from build123d import *

# Parameters (mm, degrees)
ROD_BODY_SKETCH_W                = 95
ROD_BODY_SKETCH_H                = 30
ROD_BODY_30X95_DEPTH             = 20
MOUNTING_PLATE_SKETCH_W          = 50
MOUNTING_PLATE_SKETCH_H          = 90
MOUNTING_PLATE_12MM_DEPTH        = 12
EYE_BOSS_DEPTH                   = 7.5
EYE_HOLE_SKETCH_R                = 12.5
EYE_HOLE_25_DEPTH                = 15
MOUNTING_SLOTS_2X10_DEPTH        = 138.095769446
PLATE_CORNER_CHAMFERS_10X45_SIZE = 10


with BuildPart() as part:
    # Rod Body Sketch → Rod Body 30x95 (new, symmetric)
    with BuildSketch(Plane.XY):
        Rectangle(ROD_BODY_SKETCH_W, ROD_BODY_SKETCH_H)
    extrude(amount=ROD_BODY_30X95_DEPTH, both=True)

    # Mounting Plate Sketch → Mounting Plate 12mm (add)
    with BuildSketch(Plane(origin=(0, 15, 0), x_dir=(1, 0, 0), z_dir=(0, 1, 0))):
        with Locations((-22.5, 0)):
            Rectangle(MOUNTING_PLATE_SKETCH_W, MOUNTING_PLATE_SKETCH_H)
    extrude(amount=MOUNTING_PLATE_12MM_DEPTH)

    # Eye Boss Sketch → Eye Boss (add, symmetric)
    with BuildSketch(Plane.XY):
        with BuildLine():
            Line((92.5, -15), (47.5, -15))
            Line((47.5, -15), (47.5, 15))
            Line((47.5, 15), (62.5, 15))
            ThreePointArc((62.5, 15), (113.713203436, 36.213203436), (92.5, -15))
        make_face()
    extrude(amount=EYE_BOSS_DEPTH, both=True)

    # Eye Hole Sketch → Eye Hole Ø25 (cut)
    with BuildSketch(Plane.XY.offset(7.5)):
        with Locations((92.5, 15)):
            Circle(EYE_HOLE_SKETCH_R)
    extrude(amount=-EYE_HOLE_25_DEPTH, mode=Mode.SUBTRACT)

    # Mounting Slots Sketch → Mounting Slots 2x10 (cut, through all)
    with BuildSketch(Plane(origin=(0, 27, 0), x_dir=(1, 0, 0), z_dir=(0, 1, 0))):
        with BuildLine():
            Line((-27.5, 20), (-27.5, 45))
            Line((-27.5, 45), (-17.5, 45))
            Line((-17.5, 45), (-17.5, 20))
            ThreePointArc((-17.5, 20), (-22.5, 15), (-27.5, 20))
        make_face()
        with BuildLine():
            Line((-27.5, -20), (-27.5, -45))
            Line((-27.5, -45), (-17.5, -45))
            Line((-17.5, -45), (-17.5, -20))
            ThreePointArc((-17.5, -20), (-22.5, -15), (-27.5, -20))
        make_face()
    extrude(amount=-MOUNTING_SLOTS_2X10_DEPTH, mode=Mode.SUBTRACT)

    # Plate Corner Chamfers 10x45
    plate_corner_chamfers_10x45_edges = [part.edges().sort_by_distance(p)[0] for p in [
        (-47.5, 21, -45),
        (-47.5, 21, 45),
        (2.5, 21, 45),
        (2.5, 21, -45),
    ]]
    chamfer(plate_corner_chamfers_10x45_edges, length=PLATE_CORNER_CHAMFERS_10X45_SIZE)


solid = part.part
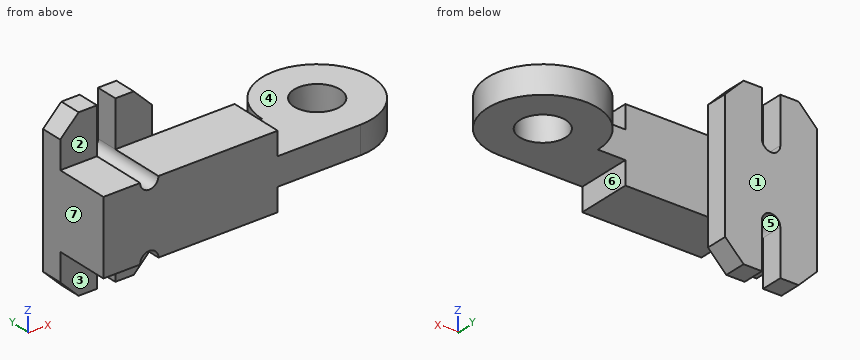
Could you check a few things on this model? Use its own coordinates, in mm. Face numbers are marked on the shaded views. A direction names the side the tool comes from. Coordinates: 2 decimals unless noted, no trailing zeros. Write each loop counter-clockwise with the first axis right and the second up, starting at its lowest first coordinate (ties: lowest second). Pieces come first, ordered by that corner, then holes. Notation, with made-up numbers: (-21.75, 59.25) - (18.25, 59.25) arc R27 ccw to (18.25, 96.25) - close; hole circle Ø7 at (74, 69). An arc over 180 degrees is marked (long way). Put each result on its own line as item: value. Start each with the question number.
Q1. I want a section at B-B on z = 27. Write out the boundary of the cut face in (x, y), plus the area to 3 significant figures.
Q2. Thinking about a two-plate mould opening in X: for the marked faces 4, 5, 6 and 7, which applies, pulls with the +X half, pulls with the -X half, needs draft (parallel to the pull), parting line crosses it, or undercut?
Q3. I'm going to push flat-ended pins straight in: P1, Ø3.5, axis at y = 21.5, z = 4, coming from the +X side; P2, Ø13, axis at y = 18, z = -36.5, coming from the +X side; P3, Ø16, axis at x = -11.5, z = -29.5, coming from the -Y side. Where does each tip first touch, or does it pass through?
Q4. I want a section at A-A on z = 2. Write out the boundary of the cut face in (x, y).
Q5. Please list where these lines run through material, in increasing order: L1, parallel to Y at x = 92.5, z = -1.5; L2, parallel to Z at x = 115, y = 33; L3, parallel to Y at x = -38, z = -39.
Q6. I want a section at D-D on y = 32. Write out the boundary of the cut face in (x, z), plus the area to 3 significant figures.
Q7. Which directions (+Z, -Z, +X, -X, +Y, -Y) give clear straight access to the entire face, cutting with the end or side of a thin tool? Please do the marked faces 1, 2 and 3.
Q8. I want a section at C-C on x = -34. Write out the boundary of the cut face in (y, z), plus the area to 3 significant figures.
Checks:
1. outline: (-47.5, 15) - (-27.5, 15) - (-27.5, 27) - (-47.5, 27) - close; (-17.5, 15) - (2.5, 15) - (2.5, 27) - (-17.5, 27) - close
1. area: 480 mm²
2. face 4: needs draft
2. face 5: undercut
2. face 6: pulls with the +X half
2. face 7: pulls with the -X half
3. P1: x = 122.12
3. P2: x = 2.5
3. P3: y = 15
4. outline: (-47.5, -15) - (92.5, -15) arc R30 ccw (long way) to (62.5, 15) - (2.5, 15) - (2.5, 27) - (-47.5, 27) - close; hole circle Ø25 at (92.5, 15)
5. L1: -15 to 2.5, 27.5 to 45
5. L2: -7.5 to 7.5
5. L3: 15 to 27
6. outline: (67.78, -7.5) - (117.22, -7.5) - (117.22, 7.5) - (67.78, 7.5) - close
6. area: 742 mm²
7. face 1: +Z, -Z, -X, +Y
7. face 2: +Z, +X, -X, -Y
7. face 3: -Z, +X, -X, -Y
8. outline: (-15, -20) - (15, -20) - (15, -45) - (27, -45) - (27, 45) - (15, 45) - (15, 20) - (-15, 20) - close
8. area: 2,280 mm²
